Input: part model. Units: mm. Frame: model coordinates. A direction names the side the tool comes from. Round coordinates to 2 decimals unless told otherwise and drop trailing zeros. Order: outer loops, then holes, each group sorted by start corner. A loop starts at its lowest first (then second) coordinate and runs counter-clockwise, first axis right, second up.
Item 1: Reachability of faces 4 (the flat face through (0, 5, -25)), 5 (the flat face through (19, 5.4, -13)) from +Z, -Z, +X, -X, +Y, -Y: full face, straight path, thin tool, end or side. Return the list, or none.
Item 2: First-contact query: pin 1 (2.5 mm diameter, centred on x = 18.5, z = -1, fed in from +Y); pin 2 (3.5 mm diameter, centred on x = 17.25, z = 0, fed in from +Y). Flat tips, straight axial feed; report the tip coordinate or a pass-through.
Item 3: Cut plane C-C on y = 1. Give the number of separate pieces and of enclosed holes in the cut face, then the cut area to 3 significant figures.
Item 4: Cut plane A-A on z = 0. Output: boundary loops of the cut face in (x, y).
Item 5: Line query: L1, parallel to Z at x = -17.25, y = 4.05; L2, parallel to Z at x = 17.25, y = 6.45; L3, parallel to Z at x = 0, y = 4.5. Output: solid intervals per line, ascending.
Item 6: Cut plane B-B on x = 0. Output: boundary loops of the cut face in (y, z).
Item 7: Cut plane D-D on z = -15. Output: boundary loops of the cut face in (x, y).
Item 8: Mould query, pull axis Z, two halves, no side actions, for faces 1 (the flat face through (0, 10, 0)), 2 (the flat face through (-22.24, 4.93, -24.01)), 3 (the cylindrical face through (14.3, 7.7, -17.7)). Classes: released by +Z, released by -Z, zero draft, split by the parting line, or undercut.
```python
from build123d import *

# Parameters (mm, degrees)
SKETCH_1_W                = 46.5
SKETCH_1_H                = 50
EXTRUDE_1_DEPTH           = 10
HOLE_WIZARD_1_D           = 4.5
HOLE_WIZARD_1_DEPTH       = 20
HOLE_WIZARD_1_CBORE_D     = 8
HOLE_WIZARD_1_CBORE_DEPTH = 4.6
HOLE_WIZARD_1_TIP         = 1.351936393
CHAMFER_1_SIZE            = 2
HOLE_WIZARD_M5_1_D        = 4.2


with BuildPart() as part:
    # 草图1 → 凸台-拉伸1 (new body)
    with BuildSketch(Plane(origin=(0, 0, 0), x_dir=(1, 0, 0), z_dir=(0, 1, 0))):
        Rectangle(SKETCH_1_W, SKETCH_1_H)
    extrude(amount=EXTRUDE_1_DEPTH)

    # 打孔尺寸(%根据)内六角圆柱头螺钉的类型1
    with Locations(Plane(origin=(0, 10, 0), x_dir=(1, 0, 0), z_dir=(0, 1, 0))):
        with Locations((17.25, -15), (17.25, 0), (17.25, 15), (-17.25, 15), (-17.25, 0), (-17.25, -15)):
            CounterBoreHole(HOLE_WIZARD_1_D / 2, HOLE_WIZARD_1_CBORE_D / 2, HOLE_WIZARD_1_CBORE_DEPTH, depth=HOLE_WIZARD_1_DEPTH)
            with Locations((0, 0, -(HOLE_WIZARD_1_DEPTH + HOLE_WIZARD_1_TIP / 2))):  # 118° drill point
                Cone(0, HOLE_WIZARD_1_D / 2, HOLE_WIZARD_1_TIP, mode=Mode.SUBTRACT)

    # 倒角1
    chamfer_1_edges = [part.edges().sort_by_distance(p)[0] for p in [
        (23.25, 5, 25),
        (-23.25, 5, 25),
        (-23.25, 5, -25),
        (23.25, 5, -25),
    ]]
    chamfer(chamfer_1_edges, length=CHAMFER_1_SIZE)

    # M5 螺纹孔1 (through all)
    with Locations(Plane(origin=(0, 10, 0), x_dir=(1, 0, 0), z_dir=(0, 1, 0))):
        with Locations((0, 15), (0, -15)):
            Hole(HOLE_WIZARD_M5_1_D / 2)


solid = part.part
```
From the geometry:
1. face 4: -Z, +X, -X, +Y, -Y
1. face 5: +Y
2. pin 1: stops at y = 5.4
2. pin 2: passes through
3. separate pieces: 1
3. enclosed holes: 8
3. area: 2,190 mm2
4. outline: (-23.25, 0) - (-19.5, 0) - (-19.5, 5.4) - (-21.25, 5.4) - (-21.25, 10) - (-23.25, 10) - close; (-15, 0) - (15, 0) - (15, 5.4) - (13.25, 5.4) - (13.25, 10) - (-13.25, 10) - (-13.25, 5.4) - (-15, 5.4) - close; (19.5, 0) - (23.25, 0) - (23.25, 10) - (21.25, 10) - (21.25, 5.4) - (19.5, 5.4) - close
5. L1: z = -25 to -17.25, -12.75 to -2.25, 2.25 to 12.75, 17.25 to 25
5. L2: z = -25 to -19, -11 to -4, 4 to 11, 19 to 25
5. L3: z = -25 to -17.1, -12.9 to 12.9, 17.1 to 25
6. outline: (0, -25) - (10, -25) - (10, -17.1) - (0, -17.1) - close; (0, -12.9) - (10, -12.9) - (10, 12.9) - (0, 12.9) - close; (0, 17.1) - (10, 17.1) - (10, 25) - (0, 25) - close
7. outline: (-23.25, 0) - (-19.5, 0) - (-19.5, 5.4) - (-21.25, 5.4) - (-21.25, 10) - (-23.25, 10) - close; (-15, 0) - (-2.1, 0) - (-2.1, 10) - (-13.25, 10) - (-13.25, 5.4) - (-15, 5.4) - close; (2.1, 0) - (15, 0) - (15, 5.4) - (13.25, 5.4) - (13.25, 10) - (2.1, 10) - close; (19.5, 0) - (23.25, 0) - (23.25, 10) - (21.25, 10) - (21.25, 5.4) - (19.5, 5.4) - close
8. face 1: zero draft
8. face 2: released by -Z
8. face 3: undercut
